```python
from build123d import *

# Parameters (mm, degrees)
BASE_PLATE_SKETCH_W             = 50
BASE_PLATE_SKETCH_H             = 90
BASE_PLATE_90X50X10_DEPTH       = 10
UPRIGHT_BLOCK_DEPTH             = 50
CYLINDRICAL_BOSS_SKETCH_R       = 20
CYLINDRICAL_BOSS_DEPTH          = 26
BOSS_SLOT_20MM_DEPTH            = 10
STEPPED_BOSS_DEPTH              = 1
STEPPED_BOSS_DEPTH_BACK         = 20
UPRIGHT_CHAMFER_10MM_SIZE       = 10
ANGLED_FACE_CUT_SKETCH_W        = 24.608073664
ANGLED_FACE_CUT_SKETCH_H        = 128.65551329
ANGLED_FACE_CUT_DEPTH           = 38
WINDOW_POCKET_SKETCH_W          = 12
WINDOW_POCKET_SKETCH_H          = 20
RECTANGULAR_WINDOW_POCKET_DEPTH = 12


with BuildPart() as part:
    # Base Plate Sketch → Base Plate 90x50x10 (new body)
    with BuildSketch(Plane(origin=(0, 0, 0), x_dir=(1, 0, 0), z_dir=(0, 1, 0))):
        with Locations((9.55801105, 0)):
            Rectangle(BASE_PLATE_SKETCH_W, BASE_PLATE_SKETCH_H)
    extrude(amount=BASE_PLATE_90X50X10_DEPTH)

    # Upright Block Sketch → Upright Block (add)
    with BuildSketch(Plane(origin=(0, 10, 0), x_dir=(1, 0, 0), z_dir=(0, 1, 0))):
        Polygon((-15.44198895, -45), (8.55801105, -45), (9.55801105, 45), (-15.44198895, 45), align=None)
    extrude(amount=UPRIGHT_BLOCK_DEPTH)

    # Cylindrical Boss Sketch → Cylindrical Boss (add)
    with BuildSketch(Plane(origin=(9.056892915, 0, 0.100632143), x_dir=(0.011110425303554966, 0, -0.9999382773199426), z_dir=(0.9999382773199426, 0, 0.011110425303554966))):
        with Locations(Location((20.103416047, 40, 0), (0, 0, 90))):
            Circle(CYLINDRICAL_BOSS_SKETCH_R)
    extrude(amount=CYLINDRICAL_BOSS_DEPTH)

    # Boss Slot Sketch → Boss Slot 20mm (cut)
    with BuildSketch(Plane(origin=(35.055288125, 0, 0.389503201), x_dir=(0.011110425303554968, 0, -0.9999382773199426), z_dir=(0.9999382773199426, 0, 0.011110425303554968))):
        with BuildLine():
            Line((10.5587389, 40), (30.5587389, 40))
            Line((30.5587389, 40), (30.5587389, 19.803393248))
            ThreePointArc((30.5587389, 19.803393248), (20.5587389, 17.463298283), (10.5587389, 19.803393248))
            Line((10.5587389, 19.803393248), (10.5587389, 40))
        make_face()
    extrude(amount=-BOSS_SLOT_20MM_DEPTH, mode=Mode.SUBTRACT)

    # Stepped Boss Sketch → Stepped Boss (add, two sides: drawn at the far end of the back side and taken through both)
    with BuildSketch(Plane(origin=(0, 60, 0), x_dir=(1, 0, 0), z_dir=(0, 1, 0)).offset(-STEPPED_BOSS_DEPTH_BACK)):
        Polygon((8.719523515, 45), (-15.44198895, 45), (-15.44198895, -5), (9.002455494, -5), (9.152545963, 8.508142185), (19.55801105, 8.508142185), (19.55801105, 36.677454153), (9.465538318, 36.677454153), (9.55801105, 45), align=None)
    extrude(amount=STEPPED_BOSS_DEPTH + STEPPED_BOSS_DEPTH_BACK)

    # Upright Chamfer 10mm
    upright_chamfer_10mm_edges = [part.edges().sort_by_distance(p)[0] for p in [
        (-3.44198895, 60, 45),
    ]]
    chamfer(upright_chamfer_10mm_edges, length=UPRIGHT_CHAMFER_10MM_SIZE)

    # Angled Face Cut Sketch → Angled Face Cut (cut)
    with BuildSketch(Plane(origin=(0, 27.701010127, 27.701010127), x_dir=(1, 0, 0), z_dir=(0, 0.7071067811865464, 0.7071067811865488))):
        with Locations((-3.137952118, -15.023583913)):
            Rectangle(ANGLED_FACE_CUT_SKETCH_W, ANGLED_FACE_CUT_SKETCH_H)
    extrude(amount=ANGLED_FACE_CUT_DEPTH, mode=Mode.SUBTRACT)

    # Window Pocket Sketch → Rectangular Window Pocket (cut)
    with BuildSketch(Plane(origin=(0, 27.701010127, 27.701010127), x_dir=(1, 0, 0), z_dir=(0, 0.7071067811865462, 0.7071067811865488))):
        with Locations((-3.44198895, 0.535533906)):
            Rectangle(WINDOW_POCKET_SKETCH_W, WINDOW_POCKET_SKETCH_H)
    extrude(amount=-RECTANGULAR_WINDOW_POCKET_DEPTH, mode=Mode.SUBTRACT)


solid = part.part
```
Check sheet for the modelled part. Datum: model origin and axes. Units: mm. A direction names the side the tool comes from. Coordinates: 2 decimals unless noted, no trailing zeros. Loops run counter-clockwise (first coordinate to the right, second up) from the corner with the lowest first, then second, coordinate; pieces in that order, holes last.
1) Sectioned sample at B-B (z = 2.5). Record the boundary of the cut face in (x, y).
2) Access from +Z, -Z, +X, -X, +Y, -Y to the whole of each face (thin tool, end or side, straight path). Record for faces 1 (the face through (2.558, 24, 23)), 2 (the face through (-1, 23, -45)), 3 (the face through (-3.526, 16.825, 30.21)).
3) Gauge pin test, flat ends, axial feed: pin 1 (25 mm diameter, centred on y = 20.5, z = 22.5, fed in from +X); pin 2 (3 mm diameter, centred on y = 36.5, z = 3.5, fed in from +X); pin 3 (8 mm diameter, centred on y = 56, z = -29, fed in from +X) (3 decimals). Record the tip position at first contact, or that the pin passes through.
4) Material ranges on probe 1 along Y at (x, z) = (10, -3); probe 2 along X at (y, z) = (4, 18); probe 3 along Y at (x, z) = (18.5, -29), recorded low to high.
5) Sectioned sample at A-A (x = 1). Record the boundary of the cut face in (y, z), and give its area (3 significant figures).
6) Sectioned sample at D-D (x = 7). Record the boundary of the cut face in (y, z).
7) Release check for a two-part mould opening along X. For faces 4 (the face through (34.558, 5, 1)), 5 (the face through (15, 56, -36.677)), 6 (the face through (22.09, 20.02, -18.98)), 7 (the face through (-15.442, 23, -11)) record: released by +X, released by -X, zero draft, split by the parting line, or undercut.
8) Sectioned sample at C-C (y = 9). Record the boundary of the cut face in (x, z), and give its area (3 significant figures).
Check sheet entries:
1. outline: (-15.44, 0) - (34.56, 0) - (34.56, 10) - (9.03, 10) - (9.03, 52.9) - (-15.44, 52.9) - close
2. face 1: none
2. face 2: -Z, +X, -X, +Y, -Y
2. face 3: +Y
3. pin 1: stops at x = 34.56
3. pin 2: stops at x = 9.04
3. pin 3: stops at x = 35.425
4. probe 1: y = 0 to 10, 29.45 to 50.55
4. probe 2: x = -15.44 to 34.56
4. probe 3: y = 0 to 10, 22.19 to 61
5. outline: (0, -45) - (61, -45) - (61, -5.6) - (35.15, 20.25) - (26.67, 11.77) - (12.52, 25.91) - (21.01, 34.39) - (10.4, 45) - (0, 45) - close
5. area: 3,970 mm2
6. outline: (0, -45) - (61, -45) - (61, -5.6) - (10.4, 45) - (0, 45) - close
7. face 4: released by +X
7. face 5: zero draft
7. face 6: undercut
7. face 7: released by -X
8. outline: (-15.44, -45) - (34.56, -45) - (34.56, 45) - (-15.44, 45) - close
8. area: 4,500 mm2
